Can you work these out from the model? Positions are in its coordinate system, mm. A direction names the side the tool comes from. Coordinates: 2 decimals unless noted, no trailing zeros. Loops run counter-clockwise (first coordinate to the right, second up) from the corner with the lowest first, then second, coordinate; pieces in that order, holes last. Notation, with made-up numbers: M 50.25,26.5 L 85.25,26.5 A26 cw 85.25,59.5 Z; hole C -36.5,47.25 d8. An arc over 180 degrees is marked long. Answer as a JSON object with one key per item and string values. Group by question number.
Item 1: We'd pull the mould along X, two halves only. Please class faces 6 (the flat face through (-1.697, -17.675, 4.93)), 7 (the flat face through (37, 52, 0)), 8 (the cylindrical face through (16.75, 32.65, 4.93)), 9 (the cylindrical face through (13.343, -21.826, 4.93)): +X half, -X half, draft (parallel to the pull), parting line (faces both ways), or undercut.
Item 2: If I drill on line 1 (Z direction, x = 38, y = 119); line 2 (Y direction, x = 0, z = 7.25); line 3 (X direction, y = 159.5, z = 4), over which ranges is the centre line in solid material (lowest first)?
Item 3: Suppose I cut it at A-A (x = 0). Write out the boundary of the cut face in (y, z), then the cut area to 3 significant figures.
Item 4: I'm going to push flat-ended pins straight in: pin 1 Ø8 at (x, z) = (28.5, -29) entering from -Y; pin 2 Ø1 at (x, z) = (44.5, -37) entering from +Y; pin 3 Ø10 at (x, y) = (29.5, -3) entering from -Z; pin 4 Ø8 at (y, z) = (78.5, 4) entering from +X. Where does each tip first touch, or does it pass through?
Item 5: Suppose I cut it at B-B (y = 82). Write out the boundary of the cut face in (x, z), then the cut area to 3 significant figures.
Item 6: Suppose I cut it at D-D (z = -48). Write out the boundary of the cut face in (x, y), then the cut area to 3 significant figures.
Item 7: Which directions (+Z, -Z, +X, -X, +Y, -Y) give clear straight access to the entire face, cutting with the end or side of a thin tool? Please do faces 1 (the cylindrical face through (19, 0, 5)), 2 (the cylindrical face through (-12.5, -0.1, 4.9)), 3 (the cylindrical face through (13.371, -32.046, 4.93)), 4 (the flat face through (41.6, 176.4, -21)), 5 (the flat face through (45, 81, 5)).
Item 8: Suppose I cut it at C-C (x = 40). Write out the boundary of the cut face in (y, z).
```python
from build123d import *

# Parameters (mm, degrees)
SKETCH_1_R      = 6
EXTRUDE_1_DEPTH = 10
SKETCH_3_R      = 7.5
EXTRUDE_2_DEPTH = 21
SKETCH_4_R      = 5
EXTRUDE_3_DEPTH = 40


with BuildPart() as part:
    # 草图1 → 凸台-拉伸1 (new body)
    with BuildSketch(Plane.XY):
        with BuildLine():
            Line((-9.678413026, 7.910646073), (6.063573898, 27.170444817))
            ThreePointArc((6.063573898, 27.170444817), (16.926727904, 32.658860626), (28.284271247, 28.284271247))
            ThreePointArc((28.284271247, 28.284271247), (32.571487227, 27.431490967), (35, 31.066017178))
            Line((35, 31.066017178), (35, 160))
            ThreePointArc((35, 160), (40, 183.956439237), (45, 160))
            Line((45, 160), (45, 0))
            ThreePointArc((45, 0), (38.630100159, -19.753777039), (21.920310217, -32.0651641))
            ThreePointArc((21.920310217, -32.0651641), (13.253400527, -32.010353988), (6.063573898, -27.170444817))
            Line((6.063573898, -27.170444817), (-9.678413026, -7.910646073))
            ThreePointArc((-9.678413026, -7.910646073), (-12.5, 0), (-9.678413026, 7.910646073))
        make_face()
        Circle(SKETCH_1_R, mode=Mode.SUBTRACT)
        with BuildLine():
            ThreePointArc((21.920310217, -21.920310217), (31, 0), (21.920310217, 21.920310217))
            ThreePointArc((21.920310217, 21.920310217), (13.435028843, 21.920310217), (13.435028843, 13.435028843))
            ThreePointArc((13.435028843, 13.435028843), (19, 0), (13.435028843, -13.435028843))
            ThreePointArc((13.435028843, -13.435028843), (13.435028843, -21.920310217), (21.920310217, -21.920310217))
        make_face(mode=Mode.SUBTRACT)
    extrude(amount=EXTRUDE_1_DEPTH)

    # 草图3 → 凸台-拉伸2 (add)
    with BuildSketch(Plane(origin=(0, 0, 0), x_dir=(-1, 0, 0), z_dir=(0, 0, -1))):
        with Locations(Location((-40, 171.456439237, 0), (0, 0, 180))):
            Circle(SKETCH_3_R)
    extrude(amount=EXTRUDE_2_DEPTH)

    # 草图4 → 凸台-拉伸3 (add)
    with BuildSketch(Plane(origin=(0, 0, -21), x_dir=(-1, 0, 0), z_dir=(0, 0, -1))):
        with Locations((-40, 171.456439237)):
            Circle(SKETCH_4_R)
    extrude(amount=EXTRUDE_3_DEPTH)


solid = part.part
```
From the geometry:
{
 "1": {"face 6": "-X half", "face 7": "draft", "face 8": "undercut", "face 9": "undercut"},
 "2": {"line 1": "0 to 10", "line 2": "-19.75 to -6, 6 to 19.75", "line 3": "35 to 45"},
 "3": {"outline": "M -19.75,0 L -6,0 L -6,10 L -19.75,10 Z; M 6,0 L 19.75,0 L 19.75,10 L 6,10 Z", "area": "275 mm2"},
 "4": {"pin 1": "through", "pin 2": "y = 174.46", "pin 3": "z = 0", "pin 4": "x = 45"},
 "5": {"outline": "M 35,0 L 45,0 L 45,10 L 35,10 Z", "area": "100 mm2"},
 "6": {"outline": "C 40,171.46 d10", "area": "78.5 mm2"},
 "7": {"face 1": "+Z, -Z", "face 2": "+Z, -Z, -X", "face 3": "+Z, -Z, -Y", "face 4": "-Z", "face 5": "+Z, -Z, +X, -Y"},
 "8": {"outline": "M -17.7,0 L 163.96,0 L 163.96,-21 L 166.46,-21 L 166.46,-61 L 176.46,-61 L 176.46,-21 L 178.96,-21 L 178.96,0 L 183.96,0 L 183.96,10 L -17.7,10 Z"}
}
